```python
from build123d import *
from build123d.topology import SkipClean

# Parameters (mm, degrees)
BRACKET_MASTER_PROFILE_SKETCH_R   = 8
BRACKET_MASTER_PROFILE_SKETCH_R_2 = 20
BASE_BLOCK_32MM_DEPTH             = 16
SKETCH1_5_W                       = 18
SKETCH1_5_H                       = 48
BORE_BOSS_BODY_64MM_DEPTH         = 64
CLEVIS_LUGS_76MM_DEPTH            = 76
LUG_PROFILE_CUT_A_DEPTH           = 142
LUG_PROFILE_CUT_B_DEPTH           = 142
SKETCH1_6_W                       = 32
SKETCH1_6_H                       = 48
PROFILE_CUT_131MM_DEPTH           = 131
SKETCH1_7_W                       = 18
SKETCH1_7_H                       = 48
PROFILE_BOSS_16MM_DEPTH           = 16
SKETCH1_15_W                      = 4
SKETCH1_15_H                      = 48
PROFILE_BOSS_32MM_DEPTH           = 16
SKETCH1_16_W                      = 4
SKETCH1_16_H                      = 48
THROUGH_CUT_147MM_DEPTH           = 147


with BuildPart() as part:
    # Bracket Master Profile Sketch → Base Block 32mm (new, symmetric)
    with BuildSketch(Plane.XY):
        with BuildLine():
            Line((-70, 56), (-70, 0))
            Line((-70, 0), (-38, 0))
            Line((-38, 0), (-38, 48))
            Line((-38, 48), (-20, 48))
            Line((-20, 48), (-16, 48))
            Line((-16, 48), (16, 48))
            Line((16, 48), (20, 48))
            Line((20, 48), (38, 48))
            Line((38, 48), (38, 0))
            Line((38, 0), (70, 0))
            Line((70, 0), (70, 56))
            ThreePointArc((70, 56), (48.056901395, 62.34853625), (37.98259606, 82.850044997))
            ThreePointArc((37.98259606, 82.850044997), (0, 122), (-37.98259606, 82.850044997))
            ThreePointArc((-37.98259606, 82.850044997), (-48.056901395, 62.34853625), (-70, 56))
        make_face()
        with Locations((-56, 14)):
            Circle(BRACKET_MASTER_PROFILE_SKETCH_R, mode=Mode.SUBTRACT)
        with Locations((-56, 42)):
            Circle(BRACKET_MASTER_PROFILE_SKETCH_R, mode=Mode.SUBTRACT)
        with Locations((56, 14)):
            Circle(BRACKET_MASTER_PROFILE_SKETCH_R, mode=Mode.SUBTRACT)
        with Locations((56, 42)):
            Circle(BRACKET_MASTER_PROFILE_SKETCH_R, mode=Mode.SUBTRACT)
        with Locations((0, 84)):
            Circle(BRACKET_MASTER_PROFILE_SKETCH_R_2, mode=Mode.SUBTRACT)
    extrude(amount=BASE_BLOCK_32MM_DEPTH, both=True)

    # Sketch1_5 → Bore Boss Body 64mm (add)
    with BuildSketch(Plane.XY):
        with Locations((-29, 24)):
            Rectangle(SKETCH1_5_W, SKETCH1_5_H)
        with Locations((29, 24)):
            Rectangle(SKETCH1_5_W, SKETCH1_5_H)
    extrude(amount=BORE_BOSS_BODY_64MM_DEPTH)

    # Clevis Lug Profile Sketch → Clevis Lugs 76mm (add)
    with BuildSketch(Plane.ZY.offset(38)):
        with BuildLine():
            ThreePointArc((64, 32), (48, 16), (64, 0))
            Line((64, 0), (64, 8))
            ThreePointArc((64, 8), (56, 16), (64, 24))
            Line((64, 24), (64, 32))
        make_face()
        with BuildLine():
            Line((64, 8), (64, 0))
            ThreePointArc((64, 0), (75.313708499, 4.686291501), (80, 16))
            ThreePointArc((80, 16), (75.313708499, 27.313708499), (64, 32))
            Line((64, 32), (64, 24))
            ThreePointArc((64, 24), (69.656854249, 21.656854249), (72, 16))
            ThreePointArc((72, 16), (69.656854249, 10.343145751), (64, 8))
        make_face()
        with BuildLine():
            ThreePointArc((64, 32), (48, 16), (64, 0))
            Line((64, 0), (64, 8))
            ThreePointArc((64, 8), (56, 16), (64, 24))
            Line((64, 24), (64, 32))
        make_face()
        with BuildLine():
            Line((64, 8), (64, 0))
            ThreePointArc((64, 0), (75.313708499, 4.686291501), (80, 16))
            ThreePointArc((80, 16), (75.313708499, 27.313708499), (64, 32))
            Line((64, 32), (64, 24))
            ThreePointArc((64, 24), (69.656854249, 21.656854249), (72, 16))
            ThreePointArc((72, 16), (69.656854249, 10.343145751), (64, 8))
        make_face()
    extrude(amount=-CLEVIS_LUGS_76MM_DEPTH)

    # Sketch2_3 → Lug Profile Cut A (cut)
    with SkipClean():  # the faces are left unmerged after this step: merging them gives an invalid solid
        with BuildSketch(Plane.ZY.offset(38)):
            with BuildLine():
                ThreePointArc((64, 24), (56, 16), (64, 8))
                Line((64, 8), (64, 16))
                Line((64, 16), (64, 24))
            make_face()
            with BuildLine():
                Line((64, 16), (64, 8))
                ThreePointArc((64, 8), (69.656854249, 10.343145751), (72, 16))
                ThreePointArc((72, 16), (69.656854249, 21.656854249), (64, 24))
                Line((64, 24), (64, 16))
            make_face()
        extrude(amount=-LUG_PROFILE_CUT_A_DEPTH, mode=Mode.SUBTRACT)

    # Sketch2_4 → Lug Profile Cut B (cut)
    with SkipClean():  # the faces are left unmerged after this step: merging them gives an invalid solid
        with BuildSketch(Plane.ZY.offset(38)):
            Polygon((16, 48), (64, 32), (64, 48), align=None)
        extrude(amount=-LUG_PROFILE_CUT_B_DEPTH, mode=Mode.SUBTRACT)

    # Sketch1_6 → Profile Cut 131mm (cut)
    with SkipClean():  # the faces are left unmerged after this step: merging them gives an invalid solid
        with BuildSketch(Plane.XY):
            with Locations((0, 24)):
                Rectangle(SKETCH1_6_W, SKETCH1_6_H)
        extrude(amount=PROFILE_CUT_131MM_DEPTH, mode=Mode.SUBTRACT)

    # Sketch1_7 → Profile Boss 16mm (add)
    with SkipClean():  # the faces are left unmerged after this step: merging them gives an invalid solid
        with BuildSketch(Plane.XY):
            with Locations((-29, 24)):
                Rectangle(SKETCH1_7_W, SKETCH1_7_H)
            with Locations((29, 24)):
                Rectangle(SKETCH1_7_W, SKETCH1_7_H)
        extrude(amount=-PROFILE_BOSS_16MM_DEPTH)

    # Sketch1_15 → Profile Boss 32mm (add, symmetric)
    with SkipClean():  # the faces are left unmerged after this step: merging them gives an invalid solid
        with BuildSketch(Plane.XY):
            with Locations((-18, 24)):
                Rectangle(SKETCH1_15_W, SKETCH1_15_H)
            with Locations((18, 24)):
                Rectangle(SKETCH1_15_W, SKETCH1_15_H)
        extrude(amount=PROFILE_BOSS_32MM_DEPTH, both=True)

    # Sketch1_16 → Through Cut 147mm (cut)
    with SkipClean():  # the faces are left unmerged after this step: merging them gives an invalid solid
        with BuildSketch(Plane.XY):
            with Locations((-18, 24)):
                Rectangle(SKETCH1_16_W, SKETCH1_16_H)
            with Locations((18, 24)):
                Rectangle(SKETCH1_16_W, SKETCH1_16_H)
        extrude(amount=THROUGH_CUT_147MM_DEPTH, mode=Mode.SUBTRACT)


solid = part.part
```
Source: CAD feature listing. Evaluate the final solid. Frame: model axes, mm. A direction names the side the tool comes from. Give positions to 0.01 mm unless a question says otherwise; leave off trailing zeros. Loops run counter-clockwise (first coordinate to the right, second up) from the corner with the lowest first, then second, coordinate; pieces in that order, holes last. Notation, with made-up numbers: (73.25, 45) -> (123.25, 45) arc R21 ccw to (123.25, 59) -> close; hole circle Ø2 at (32, 7). An arc over 180 degrees is marked (long way). Use a Markdown table: item, result. Add a question column.
(1) Section query C-C (x = -7.5). Output: boundary loops of the cut face in (y, z).
(2) Pull-direction query (X, two-part tool) for faces 1 (the face through (-20, 18, 31)), 2 (the face through (38, 18, 40)), 3 (the face through (-1, 62, 16)); classes: +X half, -X half, draft (parallel to the pull), parting line (faces both ways), or undercut.
(3) First-contact query: pin 1 Ø4.5 at (x, y) = (-18, 27) entering from +Z; pin 2 Ø1.5 at (y, z) = (74, -6.5) entering from +X; pin 3 Ø13 at (x, y) = (56, 42) entering from +Z; pin 4 Ø18.5 at (x, y) = (-56, 42) entering from +Z. Flat tips, straight axial feed; report the tip coordinate or a pass-through.
(4) Ray query, line 1 (X direction, y = 39, z = 41.5); line 2 (Y direction, x = 0, z = -8); line 3 (Y direction, x = -56, z = 2). Return the intervals inside material, ascending.
(5) Section query D-D (z = 23). Output: boundary loops of the cut face in (x, y).
(6) Section query A-A (y = 42). Output: boundary loops of the cut face in (x, z), then the cut area to 3 significant figures.
(7) Access query for faces 4 (the face through (-18, 24, 0)), 5 (the face through (16, 24, -8)), 6 (the face through (-38, 18, 40)), 7 (the face through (-62.349, 9.132, -0.224)). Directions: +Z, -Z, +X, -X, +Y, -Y. A direction counts if a zero-diameter tool reaches every point of the face in a straight line with its end or side. Return the directions, or none.
(8) Section query B-B (z = 68). Output: boundary loops of the cut face in (x, y), then the cut area to 3 significant figures.
Checked values:
| question | item | result |
|---|---|---|
| 1 | outline | (48, -16) -> (65.46, -16) -> (65.46, 16) -> (48, 16) -> close; (102.54, -16) -> (121.25, -16) -> (121.25, 16) -> (102.54, 16) -> close |
| 2 | face 1 | undercut |
| 2 | face 2 | +X half |
| 2 | face 3 | draft |
| 3 | pin 1 | z = 76.51 |
| 3 | pin 2 | x = 40.08 |
| 3 | pin 3 | through |
| 3 | pin 4 | z = 16 |
| 4 | line 1 | -38 to -20, 20 to 38 |
| 4 | line 2 | 48 to 64, 104 to 122 |
| 4 | line 3 | 0 to 6, 22 to 34, 50 to 57.65 |
| 5 | outline | (-38, 0) -> (-20, 0) -> (-20, 45.67) -> (-38, 45.67) -> close; (20, 0) -> (38, 0) -> (38, 45.67) -> (20, 45.67) -> close |
| 6 | outline | (-70, -16) -> (-64, -16) -> (-64, 16) -> (-70, 16) -> close; (-48, -16) -> (-16, -16) -> (-16, 0) -> (-20, 0) -> (-20, 34) -> (-38, 34) -> (-38, 16) -> (-48, 16) -> close; (16, -16) -> (48, -16) -> (48, 16) -> (38, 16) -> (38, 34) -> (20, 34) -> (20, 0) -> (16, 0) -> close; (64, -16) -> (70, -16) -> (70, 16) -> (64, 16) -> close |
| 6 | area | 2,950 mm^2 |
| 7 | face 4 | +Z, -Y |
| 7 | face 5 | +Z, -Z, -Y |
| 7 | face 6 | +Z, -X, +Y, -Y |
| 7 | face 7 | +Z, -Z |
| 8 | outline | (-38, 0.51) -> (-20, 0.51) -> (-20, 9.07) -> (-38, 9.07) -> close; (-38, 22.93) -> (-20, 22.93) -> (-20, 31.49) -> (-38, 31.49) -> close; (20, 0.51) -> (38, 0.51) -> (38, 9.07) -> (20, 9.07) -> close; (20, 22.93) -> (38, 22.93) -> (38, 31.49) -> (20, 31.49) -> close |
| 8 | area | 617 mm^2 |
